```python
from build123d import *

# Parameters (mm, degrees)
SKETCH1_W             = 60
SKETCH1_H             = 60
BOSS_EXTRUDE1_DEPTH   = 10
FILLET1_R             = 5
M6_TAPPED_HOLE1_D     = 5
M6_TAPPED_HOLE1_DEPTH = 15
M6_TAPPED_HOLE1_TIP   = 1.502151548
SKETCH8_R             = 2.1
CUT_EXTRUDE1_DEPTH    = 51.336896077
SKETCH9_R             = 4
CUT_EXTRUDE2_DEPTH    = 5
M4_TAPPED_HOLE1_D     = 3.3
M4_TAPPED_HOLE2_D     = 3.3


with BuildPart() as part:
    # Sketch1 → Boss-Extrude1 (new body)
    with BuildSketch(Plane.XY):
        with Locations((9.163798419, 0)):
            Rectangle(SKETCH1_W, SKETCH1_H)
    extrude(amount=BOSS_EXTRUDE1_DEPTH)

    # Fillet1
    fillet1_edges = [part.edges().sort_by_distance(p)[0] for p in [
        (-20.836201581, 30, 5),
        (39.163798419, 30, 5),
        (39.163798419, -30, 5),
        (-20.836201581, -30, 5),
    ]]
    fillet(fillet1_edges, radius=FILLET1_R)

    # M6 Tapped Hole1
    with Locations(Plane.XY.offset(10)):
        with Locations((9.163798419, -21.25), (30.814433514, 16.25), (-12.486836675, 16.25)):
            Hole(M6_TAPPED_HOLE1_D / 2, depth=M6_TAPPED_HOLE1_DEPTH)
            with Locations((0, 0, -(M6_TAPPED_HOLE1_DEPTH + M6_TAPPED_HOLE1_TIP / 2))):  # 118° drill point
                Cone(0, M6_TAPPED_HOLE1_D / 2, M6_TAPPED_HOLE1_TIP, mode=Mode.SUBTRACT)

    # Sketch8 → Cut-Extrude1 (cut, through all)
    with BuildSketch(Plane.XY.offset(10)):
        with Locations((9.163798419, 25)):
            Circle(SKETCH8_R)
        with Locations((34.163798419, 0)):
            Circle(SKETCH8_R)
        with Locations((-15.836201581, 0)):
            Circle(SKETCH8_R)
    extrude(amount=-CUT_EXTRUDE1_DEPTH, mode=Mode.SUBTRACT)

    # Sketch9 → Cut-Extrude2 (cut)
    with BuildSketch(Plane.XY.offset(10)):
        with Locations((-15.836201581, 0)):
            Circle(SKETCH9_R)
        with Locations((9.163798419, 25)):
            Circle(SKETCH9_R)
        with Locations((34.163798419, 0)):
            Circle(SKETCH9_R)
    extrude(amount=-CUT_EXTRUDE2_DEPTH, mode=Mode.SUBTRACT)

    # M4 Tapped Hole1 (through all)
    with Locations(Plane.XY.offset(10)):
        with Locations((-15.836201581, -25), (34.163798419, -25), (34.163798419, 25), (-15.836201581, 25)):
            Hole(M4_TAPPED_HOLE1_D / 2)

    # M4 Tapped Hole2 (through all)
    with Locations(Plane.XY.offset(10)):
        with Locations((9.163798419, 0)):
            Hole(M4_TAPPED_HOLE2_D / 2)


solid = part.part
```
Geometry check sheet. Reference: the model listing, model coordinates, mm. A direction names the side the tool comes from. Give positions to 0.01 mm unless a question says otherwise; leave off trailing zeros. Write each loop counter-clockwise with the first axis right and the second up, starting at its lowest first coordinate (ties: lowest second). Pieces come first, ordered by that corner, then holes.
1) Material ranges on L1, parallel to X at y = 17.5, z = 6.75; L2, parallel to Y at x = 8.5, z = 5.25; L3, parallel to X at y = -2.5, z = 8.25, recorded low to high.
2) Section check D-D, the plane y = -21.25. Record the boundary of the cut face in (x, z), and give its area (3 significant figures).
3) Access from +Z, -Z, +X, -X, +Y, -Y to the whole of each face (thin tool, end or side, straight path). Record for faces 1 (the cylindrical face through (11.167, 25.631, 2.535)), 2 (the cylindrical face through (8.643, 28.966, 7.535)).
4) Section check C-C, the plane y = 0. Record the boundary of the cut face in (x, z).
5) Section check B-B, the plane z = 5.75. State how many separate pieces and enclosed holes the cut face has, and give its area (3 significant figures).
6) Section check A-A, the plane y = 16.25. Record the boundary of the cut face in (x, z).
7) Release check for a two-part mould opening along X. For faces 3 (the cylindrical face through (-15.621, 26.636, 4.93)), 4 (the flat face through (9, -6, 10)), 5 (the cylindrical face through (-19.41, 28.496, 5.07)) record: pulls with the +X half, pulls with the -X half, needs draft (parallel to the pull), parting line crosses it, or undercut.
8) Gauge pin test, flat end, axial feed: pin 1 (5.5 mm diameter, centred on x = 34.16, y = 0, fed in from +Z). Record the tip position at first contact, or that the pin passes through.
Computed:
1. L1: x = -20.84 to -14.65, -10.32 to 28.65, 32.98 to 39.16
1. L2: y = -30 to -23.66, -18.84 to -1.51, 1.51 to 21.06, 28.94 to 30
1. L3: x = -20.84 to -18.96, -12.71 to 31.04, 37.29 to 39.16
2. outline: (-20.84, 0) - (6.66, 0) - (6.66, 10) - (-20.84, 10) - close; (11.66, 0) - (39.16, 0) - (39.16, 10) - (11.66, 10) - close
2. area: 550 mm2
3. face 1: +Z, -Z
3. face 2: +Z
4. outline: (-20.84, 0) - (-17.94, 0) - (-17.94, 5) - (-19.84, 5) - (-19.84, 10) - (-20.84, 10) - close; (-13.74, 0) - (7.51, 0) - (7.51, 10) - (-11.84, 10) - (-11.84, 5) - (-13.74, 5) - close; (10.81, 0) - (32.06, 0) - (32.06, 5) - (30.16, 5) - (30.16, 10) - (10.81, 10) - close; (36.26, 0) - (39.16, 0) - (39.16, 10) - (38.16, 10) - (38.16, 5) - (36.26, 5) - close
5. separate pieces: 1
5. enclosed holes: 11
5. area: 3,330 mm2
6. outline: (-20.84, 0) - (-14.99, 0) - (-14.99, 10) - (-20.84, 10) - close; (-9.99, 0) - (28.31, 0) - (28.31, 10) - (-9.99, 10) - close; (33.31, 0) - (39.16, 0) - (39.16, 10) - (33.31, 10) - close
7. face 3: undercut
7. face 4: needs draft
7. face 5: pulls with the -X half
8. pin 1: stops at z = 5
